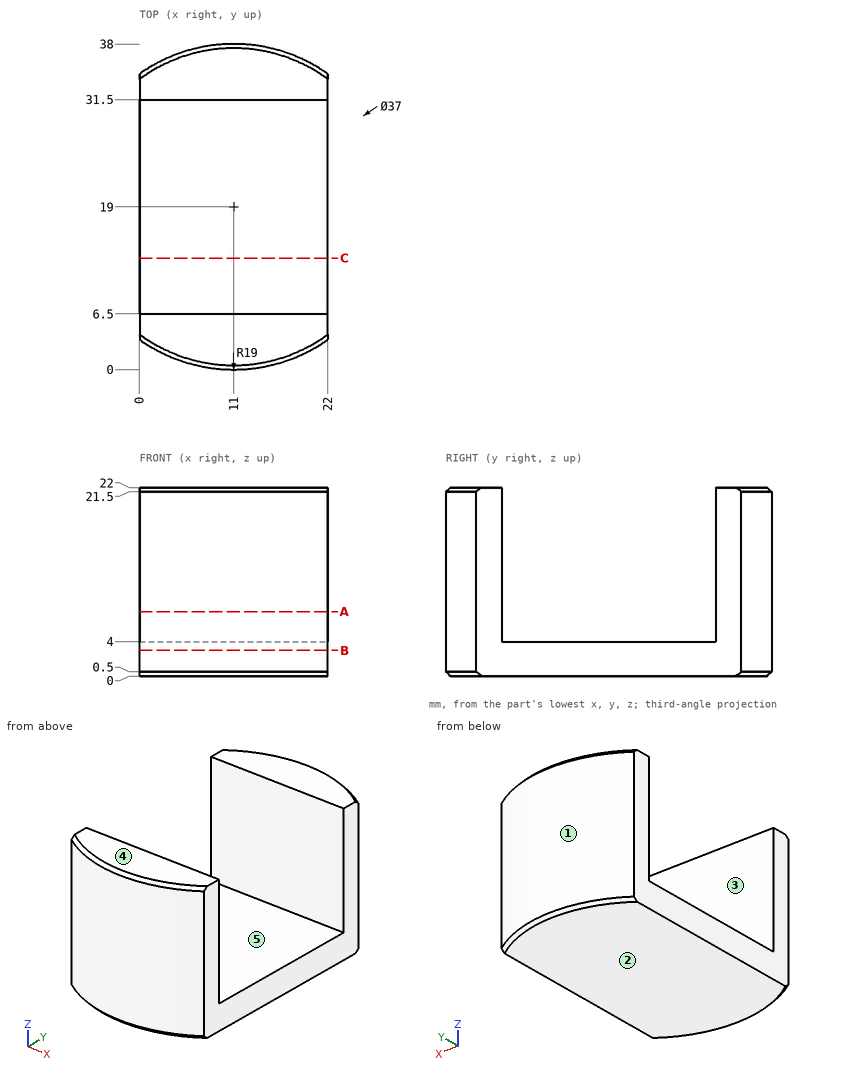
Answer from the drawing. Dimensions are ordinates in mm from the lowest x, y and z of the part. A direction names the side the tool comes from. Round coordinates to 2 decimals unless told otherwise and drop trailing zeros. Loops run counter-clockwise (first coordinate to the right, second up) from the corner with the lowest first, then second, coordinate; pieces in that order, holes last. Notation, with made-up numbers: (68, 32) - (125, 32) arc R33 cw to (125, 65) - close; hole circle Ø2 at (-10.5, -33). An arc over 180 degrees is marked (long way). One line per item, written item: value.
Q1. Each of these flat-tipped pins is pushed along its axis until it touches: pin 1 Ø10 at (y, z) = (13, 19) entering from -X; pin 2 Ø6.5 at (x, y) = (8, 20.5) entering from +Z; pin 3 Ø4 at (x, z) = (18.5, 12.5) entering from -Y; pin 4 Ø5 at (x, z) = (17.5, 14.5) entering from +Y. Where does it stop, or does it pass through?
Check values:
pin 1: through
pin 2: z = 4
pin 3: y = 0.81
pin 4: y = 37.57
Q2. Find section C-C on y = 13. Give the vertices of the cut face in (x, z), and give its area (3 significant figures).
Check values:
outline: (0, 0) - (22, 0) - (22, 4) - (0, 4) - close
area: 88.0 mm2
Q3. Find section B-B on z = 3. Give the vertices of the cut face in (x, y).
Check values:
outline: (0, 3.51) arc R19 ccw to (22, 3.51) - (22, 34.49) arc R19 ccw to (0, 34.49) - close
Q4. Straight lines are drawn through the part: probe 1 along Z at (x, y) = (6, 15.5); probe 2 along Y at (x, z) = (4.25, 9.75); probe 3 along Y at (x, z) = (15, 16.5). For each, find the intervals that lie inside material, in ascending order.
Check values:
probe 1: 0 to 4
probe 2: 1.24 to 6.5, 31.5 to 36.76
probe 3: 0.43 to 6.5, 31.5 to 37.57
Q5. For the marked faces 4 and 5, determine the directions among +Z, -Z, +X, -X, +Y, -Y from which every point of the face is accessible in a straight line to the end or side of a thin tool.
Check values:
face 4: +Z, +X, -X, +Y, -Y
face 5: +Z, +X, -X
Q6. The mould has two halves that part along Y. Classify the marked faces 1, 2 and 3: +Y half, -Y half, draft (parallel to the pull), parting line (faces both ways), or undercut.
Check values:
face 1: +Y half
face 2: draft
face 3: undercut
Q7. Find section A-A on z = 7.5. Give the vertices of the cut face in (x, y).
Check values:
outline: (0, 3.51) arc R19 ccw to (22, 3.51) - (22, 6.5) - (0, 6.5) - close; (0, 31.5) - (22, 31.5) - (22, 34.49) arc R19 ccw to (0, 34.49) - close
